```python
from build123d import *

# Parameters (mm, degrees)
BASE_PLATE_SKETCH_80X80_W          = 80
BASE_PLATE_SKETCH_80X80_H          = 80
BASE_PLATE_80X80X15_DEPTH          = 15
LOCATING_KEY_SKETCH_20X25_W        = 80
LOCATING_KEY_SKETCH_20X25_H        = 20
LOCATING_KEY_20X25X5_DEPTH         = 5
MOUNTING_HOLE_SKETCH_10_R          = 5
MOUNTING_HOLE_10_DEPTH             = 60
COUNTERBORE_SKETCH_20_R            = 10
COUNTERBORE_20X5_DEPTH             = 5
STOP_BLOCK_25_HIGH_DEPTH           = 25
V_STOP_ANGLED_FACE_CUT_30DEG_DEPTH = 100


with BuildPart() as part:
    # Base Plate Sketch 80x80 → Base Plate 80x80x15 (new body)
    with BuildSketch(Plane(origin=(0, 0, 0), x_dir=(1, 0, 0), z_dir=(0, 1, 0))):
        Rectangle(BASE_PLATE_SKETCH_80X80_W, BASE_PLATE_SKETCH_80X80_H)
    extrude(amount=BASE_PLATE_80X80X15_DEPTH)

    # Locating Key Sketch 20x25 → Locating Key 20x25x5 (add)
    with BuildSketch(Plane.XZ):
        with Locations((0, 5)):
            Rectangle(LOCATING_KEY_SKETCH_20X25_W, LOCATING_KEY_SKETCH_20X25_H)
    extrude(amount=LOCATING_KEY_20X25X5_DEPTH)

    # Mounting Hole Sketch Ø10 → Mounting Hole Ø10 (cut)
    with BuildSketch(Plane(origin=(0, 15, 0), x_dir=(1, 0, 0), z_dir=(0, 1, 0))):
        with Locations(Location((15, -5, 0), (0, 0, 270))):
            Circle(MOUNTING_HOLE_SKETCH_10_R)
    extrude(amount=-MOUNTING_HOLE_10_DEPTH, mode=Mode.SUBTRACT)

    # Counterbore Sketch Ø20 → Counterbore Ø20x5 (cut)
    with BuildSketch(Plane(origin=(0, 15, 0), x_dir=(1, 0, 0), z_dir=(0, 1, 0))):
        with Locations(Location((15, -5, 0), (0, 0, 270))):
            Circle(COUNTERBORE_SKETCH_20_R)
    extrude(amount=-COUNTERBORE_20X5_DEPTH, mode=Mode.SUBTRACT)

    # Stop Block Profile Sketch → Stop Block 25 High (add)
    with BuildSketch(Plane(origin=(0, 15, 0), x_dir=(1, 0, 0), z_dir=(0, 1, 0))):
        Polygon((40, 40), (40, 30), (25, 30), (-25, -20), (-40, -20), (-40, 40), align=None)
    extrude(amount=STOP_BLOCK_25_HIGH_DEPTH)

    # V-Stop Angle Sketch 30deg → V-Stop Angled Face Cut 30deg (cut)
    with BuildSketch(Plane(origin=(0, 0, -40), x_dir=(-1, 0, 0), z_dir=(0, 0, -1))):
        Polygon((40, 25.56624327), (15, 40), (40, 40), align=None)
    extrude(amount=-V_STOP_ANGLED_FACE_CUT_30DEG_DEPTH, mode=Mode.SUBTRACT)


solid = part.part
```
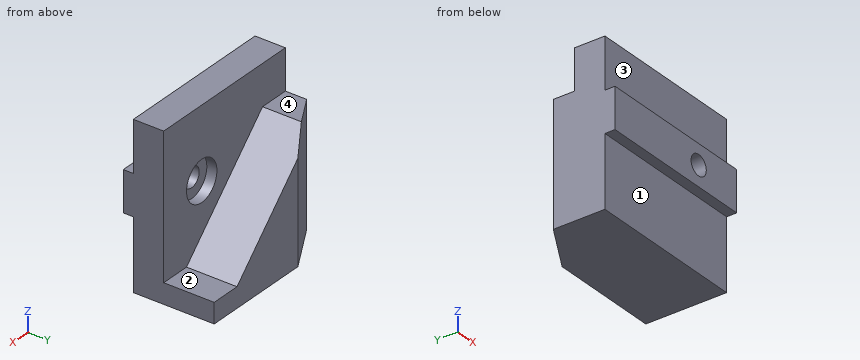
Check sheet for the modelled part. Datum: model origin and axes. Units: mm. Face numbers are marked on the shaded views. A direction names the side the tool comes from. Give positions to 0.01 mm unless a question says otherwise; leave off trailing zeros. Order: outer loops, then holes, each group sorted by start corner. A loop starts at its lowest first (then second) coordinate and runs counter-clockwise, first axis right, second up. Notation, with made-up numbers: M -5.75,1 L 18.25,1 A19 ccw 18.25,27 Z; hole C -27.75,-16.5 d5. An arc over 180 degrees is marked long. Answer in a Markdown table with one row per item. Add a question column.
Q1. Thickness scan on L1, parallel to X at y = 13, z = 5; L2, parallel to X at y = 5, z = 5; L3, parallel to Y at x = -4, z = -15.5. Record the ranges inside material, lowest first.
Q2. Sectioned sample at B-B, the plane x = 15. Record the boundary of the cut face in (y, z).
Q3. Access from +Z, -Z, +X, -X, +Y, -Y to the whole of each face (thin tool, end or side, straight path). Record for the marked faces 1, 2, 3 and 4.
Q4. Sectioned sample at A-A, the plane z = 5. Record the boundary of the cut face in (x, y), and give its area (3 significant figures).
Q5. Sectioned sample at D-D, the plane y = 13. Record the boundary of the cut face in (x, z), and give its area (3 significant figures).
Q6. Sectioned sample at C-C, the plane z = -24. Record the boundary of the cut face in (x, y).
Q7. Gauge pin test, flat ends, axial feed: pin 1 Ø13 at (x, z) = (15, 5) entering from -Y; pin 2 Ø4.5 at (x, y) = (-35, 24.5) entering from +Z; pin 3 Ø2.5 at (x, y) = (17, -3.5) entering from +Z; pin 4 Ø16.5 at (x, y) = (32.5, 28) entering from +Z. Record the tip position at first contact, or that the pin passes through.
Verdict:
| question | item | result |
|---|---|---|
| 1 | L1 | -40 to 5, 25 to 40 |
| 1 | L2 | -40 to 10, 20 to 40 |
| 1 | L3 | 0 to 40 |
| 2 | outline | M -5,-5 L 0,-5 L 0,-40 L 40,-40 L 40,-20 L 15,-20 L 15,-5 L 10,-5 L 10,0 L -5,0 Z; M -5,10 L 10,10 L 10,15 L 15,15 L 15,40 L 0,40 L 0,15 L -5,15 Z |
| 3 | face 1 | -Z, +X, -X, -Y |
| 3 | face 2 | +Z, +X, +Y |
| 3 | face 3 | +Z, +X, -X, -Y |
| 3 | face 4 | +Z, +X, -X, +Y |
| 4 | outline | M -40,-5 L 10,-5 L 10,10 L 5,10 L 5,15 L -10,15 L -10,40 L -15,40 L -40,25.57 Z; M 20,-5 L 40,-5 L 40,15 L 25,15 L 25,10 L 20,10 Z |
| 4 | area | 1,920 mm² |
| 5 | outline | M -40,-40 L 40,-40 L 40,40 L -40,40 Z; hole C 15,5 d20 |
| 5 | area | 6,090 mm² |
| 6 | outline | M -40,0 L 40,0 L 40,15 L 19,15 L 19,40 L -15,40 L -40,25.57 Z |
| 7 | pin 1 | y = -5 |
| 7 | pin 2 | z = 20 |
| 7 | pin 3 | z = 15 |
| 7 | pin 4 | z = -29.25 |
